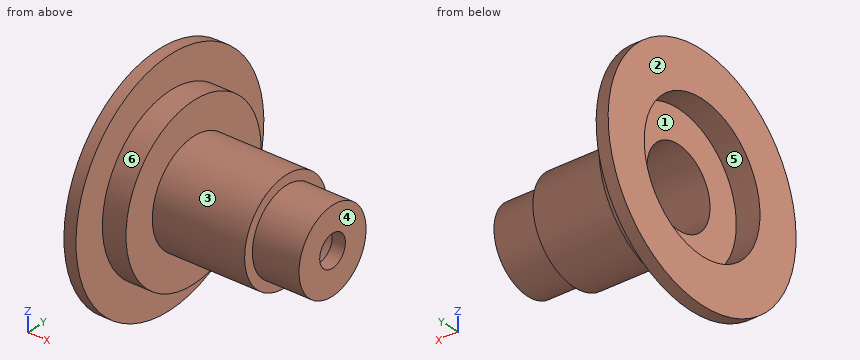
from build123d import *


with BuildPart() as part:
    # Sketch1 → Revolve1 (revolve)
    with BuildSketch(Plane.XY, mode=Mode.PRIVATE) as revolve1_sk:
        Polygon((74.14259961, 24.279053073), (74.14259961, 17.45458405), (79.060819611, 17.45458405), (79.060819611, 10.659632807), (98.286326817, 10.659632807), (98.286326817, 8.659632807), (108, 8.659632807), (108, 3.313609887), (105.27792564, 3.313609887), (105.27792564, 6.159632807), (95.786326817, 6.159632807), (95.786326817, 8.159632807), (76.560819611, 8.159632807), (76.560819611, 14.95458405), (71.64259961, 14.95458405), (71.64259961, 24.279053073), align=None)
    revolve(revolve1_sk.sketch.rotate(Axis((0, 0, 0), (-1, 0, 0)), 90), axis=Axis((0, 0, 0), (-1, 0, 0)))


solid = part.part
Here's how the part is built. I have some questions about the finished solid (model axes, mm). Face numbers are marked on the shaded views. A direction names the side the tool comes from. Round coordinates to 2 decimals unless told otherwise and drop trailing zeros. Order: outer loops, then holes, each group sorted by start corner. A loop starts at its lowest first (then second) coordinate and runs counter-clockwise, first axis right, second up. Notation, with made-up numbers: M 1.5,46 L 44.5,46 A16 ccw 44.5,55 Z; hole C 63,39.5 d4. An arc over 180 degrees is marked long. One line per question, with ' | ' between items.
1) Imagine slicing it at C-C, the plane x = 77.5. Write out the boundary of the cut face in (y, z).
Checked values:
outline: C 0,0 d34.91; hole C 0,0 d16.32
2) I need wall thicknesses on line 1 (Y direction, x = 72.75, z = 0); line 2 (Y direction, x = 107, z = 0); line 3 (X direction, y = 11.5, z = 7). Which ranges of each line are inside material? Lowest first, please.
Checked values:
line 1: y = -24.28 to -14.95, 14.95 to 24.28 | line 2: y = -8.66 to -3.31, 3.31 to 8.66 | line 3: x = 76.56 to 79.06
3) Imagine slicing it at D-D, the plane z = -13.5. Write out the boundary of the cut face in (x, y).
Checked values:
outline: M 71.64,-20.18 L 74.14,-20.18 L 74.14,-11.06 L 79.06,-11.06 L 79.06,11.06 L 74.14,11.06 L 74.14,20.18 L 71.64,20.18 L 71.64,6.43 L 76.56,6.43 L 76.56,-6.43 L 71.64,-6.43 Z
4) We'd pull the mould along Y, two halves only. Please class the marked faces 1, 2 and 3: released by +Y, released by -Y, zero draft, split by the parting line, or undercut.
Checked values:
face 1: undercut | face 2: zero draft | face 3: split by the parting line
5) On a 3-axis mill with a long thin cutter (end or side, diameter ignored), from which of +Z, -Z, +X, -X, +Y, -Y can I reach the whole of each face in a straight line? I mean the marked faces 4, 5 and 6. Say none if no direction works.
Checked values:
face 4: +Z, -Z, +X, +Y, -Y | face 5: -X | face 6: +X
6) I'm going to push flat-ended pins straight in: pin 1 Ø13 at (y, z) = (-3, -3.5) entering from -X; pin 2 Ø4 at (x, z) = (86.5, -10.5) entering from -Y; pin 3 Ø6 at (x, y) = (91.5, -12.5) entering from +Z. Where does each tip first touch, or does it pass through?
Checked values:
pin 1: stops at x = 76.56 | pin 2: stops at y = -6.43 | pin 3: stops at z = 4.84
